Source: three-view drawing plus pictorial views. Frame: mm from the lowest corner of the part. A direction names the side the tool comes from. Coordinates: 2 decimals unless noted, no trailing zeros. Order: outer loops, then holes, each group sorted by start corner. A loop starts at its lowest first (then second) coordinate and runs counter-clockwise, first axis right, second up. Notation, with made-up numbers: (12.25, 74.25) - (34.25, 74.25) arc R21 ccw to (34.25, 85.25) - close; hole circle Ø5 at (-14.5, 59.5). An arc over 180 degrees is marked (long way). One line per question, with ' | ' between items.
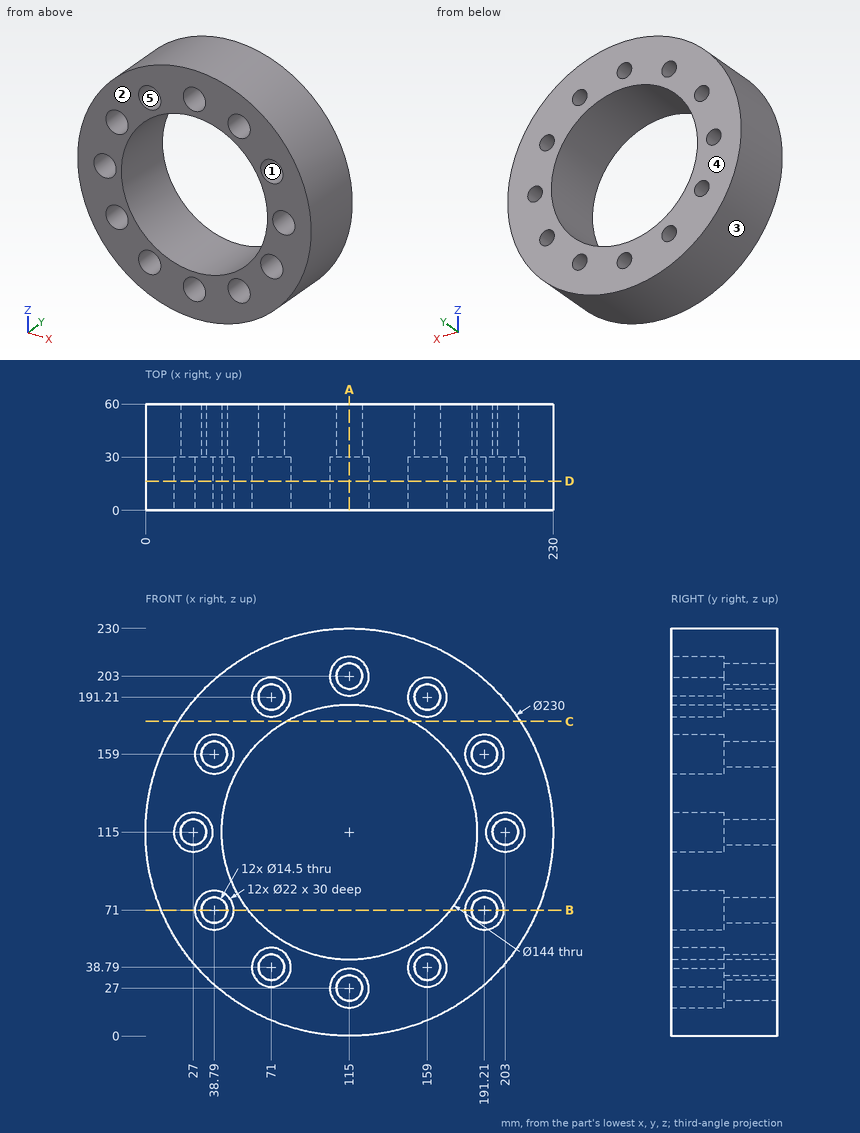
(1) Cut plane A-A (x = 115). Return the cut outline in (y, z).
Taken from the geometry:
outline: (0, 0) - (60, 0) - (60, 19.75) - (30, 19.75) - (30, 16) - (0, 16) - close; (0, 38) - (30, 38) - (30, 34.25) - (60, 34.25) - (60, 43) - (0, 43) - close; (0, 187) - (60, 187) - (60, 195.75) - (30, 195.75) - (30, 192) - (0, 192) - close; (0, 214) - (30, 214) - (30, 210.25) - (60, 210.25) - (60, 230) - (0, 230) - close
(2) Material intervals for L1, parallel to X at y = 38, z = 116.5 (1 decimal); L2, parallel to X at y = 6.5, z = 105 (1 decimal); L3, parallel to Z at x = 156, y = 24, sorted ascending. Write a range as from..to.
Taken from the geometry:
L1: x = 0..19.9, 34.1..43, 187..195.9, 210.1..230 | L2: x = 0.4..22.4, 31.6..43.7, 186.3..198.4, 207.6..229.6 | L3: z = 7.56..28.21, 49.37..55.81, 174.19..180.63, 201.79..222.44
(3) Cut plane D-D (y = 16.5). State how many separate pieces and enclosed holes the cut face has, and give its area (3 significant figures).
Taken from the geometry:
separate pieces: 1 | enclosed holes: 13 | area: 20,700 mm²
(4) Cut plane B-B (z = 71). Return the cut outline in (x, y), and give its area (3 significant figures).
Taken from the geometry:
outline: (8.75, 0) - (27.79, 0) - (27.79, 30) - (31.54, 30) - (31.54, 60) - (8.75, 60) - close; (46.04, 30) - (49.79, 30) - (49.79, 0) - (58.01, 0) - (58.01, 60) - (46.04, 60) - close; (171.99, 0) - (180.21, 0) - (180.21, 30) - (183.96, 30) - (183.96, 60) - (171.99, 60) - close; (198.46, 30) - (202.21, 30) - (202.21, 0) - (221.25, 0) - (221.25, 60) - (198.46, 60) - close | area: 3,720 mm²
(5) Set-up query: the marked faces 4 and 5. Return all of +Z, -Z, +X, -X, +Y, -Y with unobstructed straight access to the full face (end or side cutting, diameter ignored); none if empty.
Taken from the geometry:
face 4: +Z, -Z, +X, -X, +Y | face 5: -Y
(6) Pull-direction query (Z, two-part tool) for the marked faces 1, 2 and 3; classes: pulls with the +Z half, pulls with the -Z half, needs draft (parallel to the pull), parting line crosses it, or undercut.
Taken from the geometry:
face 1: undercut | face 2: needs draft | face 3: parting line crosses it
(7) Cut plane C-C (z = 177.5). Return the cut outline in (x, y), and give its area (3 significant figures).
Taken from the geometry:
outline: (18.47, 0) - (79.25, 0) - (79.25, 60) - (18.47, 60) - close; (150.75, 0) - (211.53, 0) - (211.53, 60) - (150.75, 60) - close | area: 7,290 mm²
(8) Pin query (flat end, axial travel): P1, Ø20, axis at x = 38.79, z = 159, coming from the -Y side; P2, Ø2, axis at x = 192, y = 52.5, coming from the +Z side; P3, Ø17.5, axis at x = 159, z = 191.21, coming from the +Y side; P4, Ø2, axis at y = 13, z = 95, coming from the -X side. Return the tip coordinate at first contact, or that it passes through.
Taken from the geometry:
P1: stops at y = 30 | P2: stops at z = 201.31 | P3: stops at y = 60 | P4: stops at x = 1.58
